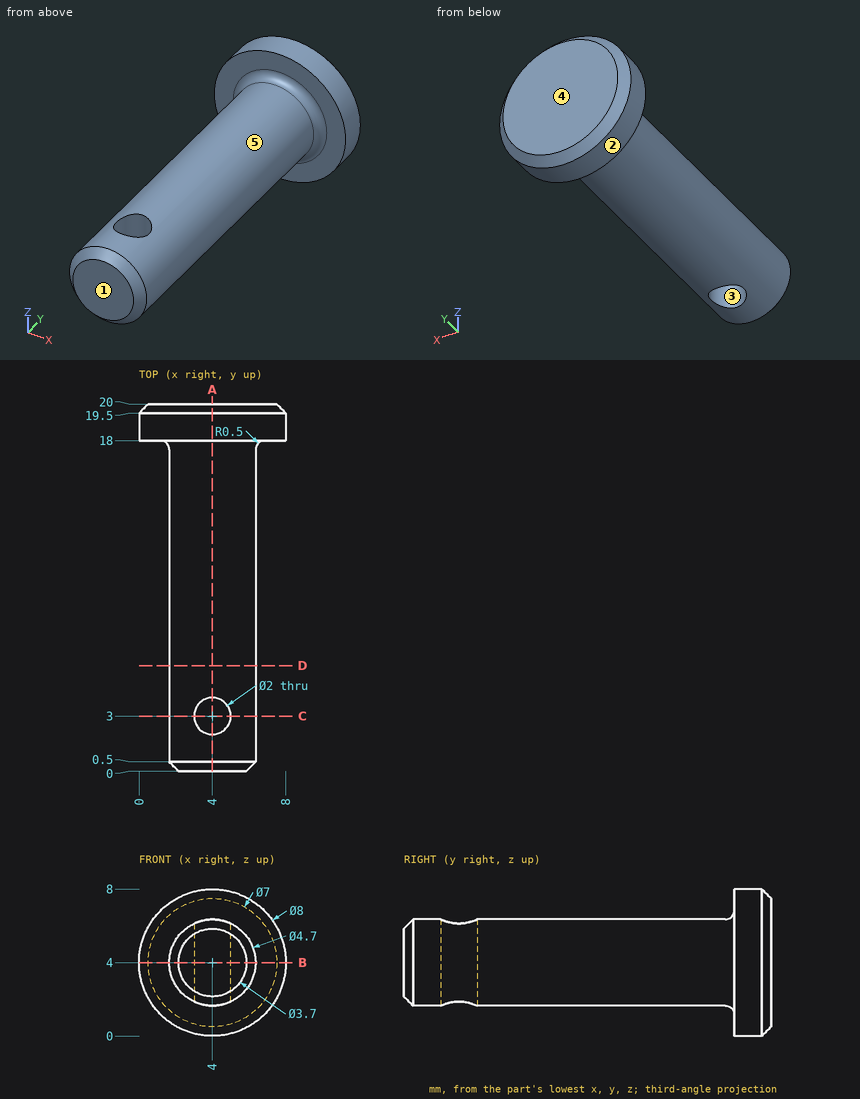
Could you check a few things on this drawing? It's one solid part, dimensions in mm from its lowest x, y, z. A direction names the side the tool comes from. Round coordinates to 2 decimals unless told otherwise and drop trailing zeros. Loops run counter-clockwise (first coordinate to the right, second up) from the corner with the lowest first, then second, coordinate; pieces in that order, holes last. Notation, with made-up numbers: (26, -30.5) -> (79, -30.5) arc R13 cw to (79, -23.5) -> close; hole circle Ø5 at (-24, 13.5). An arc over 180 degrees is marked (long way). Answer as CSV lines item,"result".
1. If we section it at D-D on y = 5.75: Please give me the cut outline in (x, z).
Final values:
outline,"circle Ø4.7 at (4, 4)"
2. If we section it at A-A on x = 4: Please give me the cut outline in (y, z), plus the area to 3 significant figures.
Final values:
outline,"(0, 2.15) -> (0.5, 1.65) -> (2, 1.65) -> (2, 6.35) -> (0.5, 6.35) -> (0, 5.85) -> close; (4, 1.65) -> (17.5, 1.65) arc R0.5 cw to (18, 1.15) -> (18, 0) -> (19.5, 0) -> (20, 0.5) -> (20, 7.5) -> (19.5, 8) -> (18, 8) -> (18, 6.85) arc R0.5 cw to (17.5, 6.35) -> (4, 6.35) -> close"
area,"90.8 mm^2"
3. Which directions (+Z, -Z, +X, -X, +Y, -Y) give clear straight access to the entire face, cutting with the end or side of a thin tool? Please do the marked faces 4 and 5.
Final values:
face 4,"+Z, -Z, +X, -X, +Y"
face 5,"-Y"
4. If we section it at C-C on y = 3: Please give me the cut outline in (x, z).
Final values:
outline,"(3, 1.87) -> (3, 6.13) arc R2.35 ccw to start; (5, 1.87) arc R2.35 ccw to (5, 6.13) -> close"
5. For pin 1 (1.5 mm diameter, centred on y = 6, z = 1.5, fed in from -X); pin 2 (4 mm diameter, centred on x = 6.5, y = 3, fed in from +Z); pin 3 (1.5 mm diameter, centred on x = 3, y = 7.5, fed in from -Z), each with a flat end and sliding along its axis, tell me the tip position at first contact or that it passes through.
Final values:
pin 1,"stops at x = 2.43"
pin 2,"stops at z = 6.26"
pin 3,"stops at z = 1.66"
6. If I drill on L1, parallel to Y at x = 4, z = 4.8; L2, parallel to Z at x = 4, y = 16.25; L3, parallel to Y at x = 4.5, z = 6, over which ranges is the centre line in solid material (lowest first)?
Final values:
L1,"y = 0 to 2, 4 to 20"
L2,"z = 1.65 to 6.35"
L3,"y = 0.21 to 2.13, 3.87 to 20"
7. Thinking about a two-plate mould opening in X: for the marked faces 1, 2 and 3, which applies, released by +X, released by -X, zero draft, split by the parting line, or undercut?
Final values:
face 1,"zero draft"
face 2,"split by the parting line"
face 3,"undercut"
8. If we section it at B-B on z = 4: Please give me the cut outline in (x, y).
Final values:
outline,"(0, 18) -> (1.15, 18) arc R0.5 cw to (1.65, 17.5) -> (1.65, 0.5) -> (2.15, 0) -> (5.85, 0) -> (6.35, 0.5) -> (6.35, 17.5) arc R0.5 cw to (6.85, 18) -> (8, 18) -> (8, 19.5) -> (7.5, 20) -> (0.5, 20) -> (0, 19.5) -> close; hole circle Ø2 at (4, 3)"
